from build123d import *

# Parameters (mm, degrees)
DOME_SLOT_CUT_DEPTH = 105
ANGLED_CUT_SKETCH_R = 75
ANGLED_CUT_DEPTH    = 75
ANGLED_CUT_DRAFT    = -39
TUBE_BORE_SKETCH_R  = 20
TUBE_BORE_CUT_DEPTH = 75
TUBE_FILLET_R5_R    = 5


with BuildPart() as part:
    # Dome Profile Sketch → Dome R80 (revolve)
    with BuildSketch(Plane.XY):
        with BuildLine():
            Line((0, 0), (0, 80))
            ThreePointArc((0, 80), (56.568542495, 56.568542495), (80, 0))
            Line((80, 0), (0, 0))
        make_face()
    revolve(axis=Axis((0, 0, 0), (0, 1, 0)))

    # Dome Slot Sketch → Dome Slot Cut (cut, symmetric)
    with BuildSketch(Plane(origin=(0, 0, 0), x_dir=(0, 0, -1), z_dir=(1, 0, 0))):
        Polygon((5, 75), (5, 5), (-5, 5), (-5, 75), (-5, 78), (-5, 79), (-5, 79.5), (5, 79.5), (5, 78), align=None)
    extrude(amount=DOME_SLOT_CUT_DEPTH, both=True, mode=Mode.SUBTRACT)


with BuildPart() as angled_cut_tool:
    # Angled Cut Sketch → Angled Cut (with draft: the straight prism first)
    with BuildSketch(Plane.XZ):
        Circle(ANGLED_CUT_SKETCH_R)
    extrude(amount=-ANGLED_CUT_DEPTH)
    # Angled Cut: the draft: its side faces are tilted about the plane it starts from
    angled_cut_sides = [angled_cut_tool.faces().sort_by_distance(p)[0] for p in [
        (-75, 37.5, 0),
    ]]
    draft(angled_cut_sides, Plane.XZ, ANGLED_CUT_DRAFT)


with BuildPart() as part_1:
    add(part.part)

    # Angled Cut: cut by angled_cut_tool
    add(angled_cut_tool.part, mode=Mode.SUBTRACT)

    # Tube Boss Profile Sketch → Tube Boss (revolve)
    with BuildSketch(Plane(origin=(0, 0, 0), x_dir=(0, 0, -1), z_dir=(1, 0, 0))):
        Polygon((47.694291303, 47.694291303), (84.852813742, 84.852813742), (106.066017178, 63.639610307), (68.907494738, 26.481087867), (50.800202422, 44.588380184), align=None)
    tube_boss = revolve(axis=Axis((0, 47.694291303, -47.694291303), (0, 0.7071067811865478, -0.7071067811865474)))

    # Tube Bore Sketch → Tube Bore Cut (cut)
    with BuildSketch(Plane(origin=(0, 84.852813742, -84.852813742), x_dir=(1, 0, 0), z_dir=(0, 0.7071067811865477, -0.7071067811865475))):
        with Locations(Location((0, 0, 0), (0, 0, 270))):
            Circle(TUBE_BORE_SKETCH_R)
    tube_bore_cut = extrude(amount=-TUBE_BORE_CUT_DEPTH, mode=Mode.SUBTRACT)

    # Tube Bore Mirror: Tube Boss, Tube Bore Cut across plane
    add(tube_boss.mirror(Plane.XY))
    add(tube_bore_cut.mirror(Plane.XY), mode=Mode.SUBTRACT)

    # Tube Fillet R5
    tube_fillet_r5_edges = [part_1.edges().sort_by_distance(p)[0] for p in [
        (0, 73.653645844, -31.227238973),
        (0, 73.653645844, 31.227238973),
    ]]
    fillet(tube_fillet_r5_edges, radius=TUBE_FILLET_R5_R)


solid = part_1.part
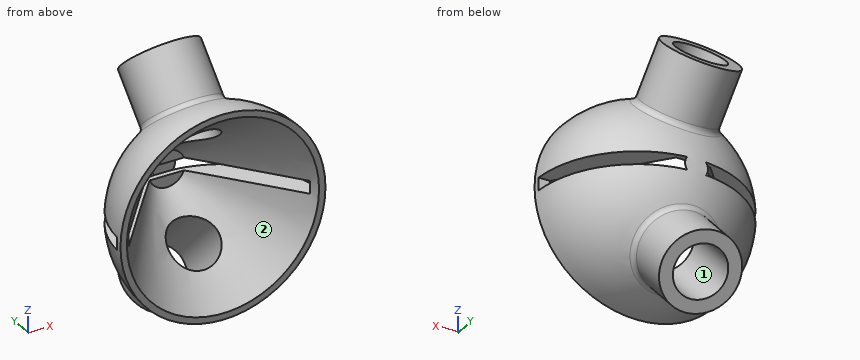
Model file for the job. Use its own axes, mm. Face numbers are marked on the shaded views. Coordinates: 2 decimals unless noted, no trailing zeros. Order: outer loops, then holes, each group sorted by start corner. A loop starts at its lowest first (then second) coordinate and runs counter-clockwise, first axis right, second up. Notation, with made-up numbers: (2, -30) -> (27, -30) arc R21 ccw to (27, 2) -> close; hole circle Ø9 at (12, 4.25). An arc over 180 degrees is marked (long way). Return JSON: item names as keys, results as strings. Group by question number.
Item 1: Pull direction Y, two halves, no side cores. Call the marked faces 1 and 2: pulls with the +Y half, pulls with the -Y half, needs draft (parallel to the pull), parting line crosses it, or undercut.
Item 2: Wall check: line 1 along Z through (x, y) = (7.5, 69.5); line 2 along Z through (x, y) = (6.5, 4.5); line 3 along X through (y, z) = (62, 46). Give the ranges that are in metal, low to high. Write a range as [from, to].
Item 3: Saw through at C-C on x = 0. State how many separate pieces and enclosed holes the cut face has, then the cut area to 3 significant figures.
Item 4: Flat gauge pins, fed straight in: P1, Ø3, axis at x = -1.5, z = -2, coming from the -Y side; P2, Ø4.5, axis at x = 77.5, z = 2.5, coming from the +Y side; P3, Ø5, axis at x = 61, z = 40, coming from the -Y side; P4, Ø10, axis at x = 1, z = -12, coming from the -Y side. Where does each tip first touch, or does it go through?
Item 5: Saw through at A-A on z = 0. Write the cut outline in (x, y).
Values found:
{
 "1": {"face 1": "undercut", "face 2": "pulls with the -Y half"},
 "2": {"line 1": "z = [-100.21, -95.72], [-43.28, -17.15], [17.15, 43.28], [95.72, 100.21]", "line 2": "z = [-79.61, -71.06], [71.06, 79.61]", "line 3": "x = [-27.92, -16.49], [16.49, 27.92]"},
 "3": {"separate pieces": "3", "enclosed holes": "0", "area": "3,440 mm2"},
 "4": {"P1": "stops at y = 79.5", "P2": "stops at y = 5", "P3": "stops at y = 0", "P4": "stops at y = 71.57"},
 "5": {"outline": "(-80, 0) -> (-75, 0) -> (-70.95, 5) -> (-79.84, 5) arc R80 ccw to start; (-8.93, 79.5) -> (8.93, 79.5) arc R80 ccw to start; (70.95, 5) -> (75, 0) -> (80, 0) arc R80 ccw to (79.84, 5) -> close"}
}
